Can you work these out from the model? Positions are in its coordinate system, mm. Give positions to 0.01 mm unless a question says otherwise; leave off trailing zeros. Loops run counter-clockwise (first coordinate to the right, second up) from the corner with the lowest first, then second, coordinate; pieces in that order, holes last. Notation, with made-up numbers: (1.25, 25.5) - (13.25, 25.5) arc R20 ccw to (13.25, 31.5) - close; hole circle Ø10 at (-4, 67.25). An arc over 180 degrees is marked (long way). Answer in a Markdown table with one row per item.
from build123d import *

# Parameters (mm, degrees)
SKETCH_1_W      = 174
SKETCH_1_H      = 136
SKETCH_1_R      = 16
SKETCH_1_W_2    = 5
SKETCH_1_H_2    = 12.5
EXTRUDE_1_DEPTH = 12
FILLET_2_R      = 10


with BuildPart() as part:
    # 草图1 → 凸台-拉伸1 (new body)
    with BuildSketch(Plane.XY):
        with Locations((-22.664999192, 1.659931171)):
            Rectangle(SKETCH_1_W, SKETCH_1_H)
        with Locations((-89.664999192, 49.659931171)):
            Circle(SKETCH_1_R, mode=Mode.SUBTRACT)
        with Locations(Location((44.335000808, 49.659931171, 0), (0, 0, 180))):
            Circle(SKETCH_1_R, mode=Mode.SUBTRACT)
        with Locations((-40.414999192, 16.852464835)):
            Rectangle(SKETCH_1_W_2, SKETCH_1_H_2, mode=Mode.SUBTRACT)
        with Locations((-40.414999192, -6.897535165)):
            Rectangle(SKETCH_1_W_2, SKETCH_1_H_2, mode=Mode.SUBTRACT)
        with Locations((-40.414999192, -30.647535165)):
            Rectangle(SKETCH_1_W_2, SKETCH_1_H_2, mode=Mode.SUBTRACT)
        with Locations((-4.914999192, -30.647535165)):
            Rectangle(SKETCH_1_W_2, SKETCH_1_H_2, mode=Mode.SUBTRACT)
        with Locations((-4.914999192, -6.897535165)):
            Rectangle(SKETCH_1_W_2, SKETCH_1_H_2, mode=Mode.SUBTRACT)
        with Locations((-4.914999192, 16.852464835)):
            Rectangle(SKETCH_1_W_2, SKETCH_1_H_2, mode=Mode.SUBTRACT)
    extrude(amount=EXTRUDE_1_DEPTH)

    # 圆角2
    fillet_2_edges = [part.edges().sort_by_distance(p)[0] for p in [
        (64.335000808, 69.659931171, 6),
        (-109.664999192, 69.659931171, 6),
    ]]
    fillet(fillet_2_edges, radius=FILLET_2_R)


solid = part.part
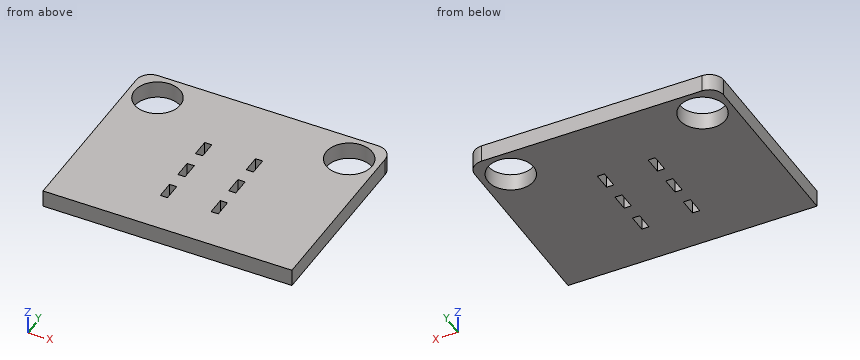
Q1. If I drill on line 1 (Y direction, x = -41.5, z = 4.25); line 2 (X direction, y = 16, z = 2.75) (3 decimals); line 3 (X direction, y = 39, z = 2.25) (3 decimals), over which ranges is the centre line in solid material (lowest first)? Write a range as [from, to].
Checked values:
| item | result |
|---|---|
| line 1 | y = [-66.34, -36.9], [-24.4, -13.15], [-0.65, 10.6], [23.1, 69.66] |
| line 2 | x = [-109.665, -42.915], [-37.915, -7.415], [-2.415, 64.335] |
| line 3 | x = [-109.665, -101.597], [-77.733, 32.403], [56.267, 64.335] |
Q2. Imagine slicing it at B-B, the plane z = 10. Count the separate pieces of the cut face and the enclosed holes in it, and give its area (3 significant figures).
Checked values:
| item | result |
|---|---|
| separate pieces | 1 |
| enclosed holes | 8 |
| area | 21,600 mm² |
Q3. Imagine slicing it at C-C, the plane y = 53.5. Write out the boundary of the cut face in (x, z) (3 decimals), and give its area (3 significant figures).
Checked values:
| item | result |
|---|---|
| outline | (-109.665, 0) - (-105.197, 0) - (-105.197, 12) - (-109.665, 12) - close; (-74.133, 0) - (28.803, 0) - (28.803, 12) - (-74.133, 12) - close; (59.867, 0) - (64.335, 0) - (64.335, 12) - (59.867, 12) - close |
| area | 1,340 mm² |
Q4. Imagine slicing it at D-D, the plane x = -80.5. Write out the boundary of the cut face in (y, z).
Checked values:
| item | result |
|---|---|
| outline | (-66.34, 0) - (36.54, 0) - (36.54, 12) - (-66.34, 12) - close; (62.77, 0) - (69.66, 0) - (69.66, 12) - (62.77, 12) - close |
Q5. Imagine slicing it at A-A, the plane x = 34. Write out the boundary of the cut face in (y, z).
Checked values:
| item | result |
|---|---|
| outline | (-66.34, 0) - (37.45, 0) - (37.45, 12) - (-66.34, 12) - close; (61.87, 0) - (69.66, 0) - (69.66, 12) - (61.87, 12) - close |
